Geometry: final body of the model. Coordinates: model frame, mm. A direction names the side the tool comes from. Give positions to 0.01 mm unless a question says otherwise; leave off trailing zeros. Order: outer loops, then holes, each group sorted by start corner. A loop starts at its lowest first (then second) coordinate and runs counter-clockwise, first axis right, second up. Notation, with made-up numbers: (-35.75, -19) - (17.25, -19) arc R14 cw to (17.25, -4) - close; hole circle Ø4 at (16, -9.5). An arc over 180 degrees is marked (long way). One line per item, written item: value.
```python
from build123d import *

# Parameters (mm, degrees)
SKETCH_1_W          = 80
SKETCH_1_H          = 50
EXTRUDE_1_DEPTH     = 1000
FILLET_1_R          = 5
SHELL_1_T           = -3
SKETCH_2_R          = 17.6
CUT_EXTRUDE_1_DEPTH = 1003.047903047
SKETCH_3_R          = 3.4
CUT_EXTRUDE_2_DEPTH = 10
SKETCH_4_R          = 2.5
CUT_EXTRUDE_3_DEPTH = 10


with BuildPart() as part:
    # 草图1 → 凸台-拉伸1 (new body)
    with BuildSketch(Plane.XY):
        Rectangle(SKETCH_1_W, SKETCH_1_H)
    extrude(amount=EXTRUDE_1_DEPTH)

    # 圆角1
    fillet_1_edges = [part.edges().sort_by_distance(p)[0] for p in [
        (40, -25, 500),
        (-40, -25, 500),
        (-40, 25, 500),
        (40, 25, 500),
    ]]
    fillet(fillet_1_edges, radius=FILLET_1_R)

    # 抽壳1
    shell_1_openings = [part.faces().sort_by_distance(p)[0] for p in [
        (0, 0, 1000),
        (0, 0, 0),
    ]]
    offset(amount=SHELL_1_T, openings=shell_1_openings, kind=Kind.INTERSECTION)

    # 草图2 → 切除-拉伸1 (cut, through all)
    with BuildSketch(Plane(origin=(0, 25, 0), x_dir=(1, 0, 0), z_dir=(0, 1, 0))):
        with Locations(Location((-4.7, -208, 0), (0, 0, 270))):
            Circle(SKETCH_2_R)
        with Locations(Location((-4.7, -792, 0), (0, 0, 270))):
            Circle(SKETCH_2_R)
    extrude(amount=-CUT_EXTRUDE_1_DEPTH, mode=Mode.SUBTRACT)

    # 草图3 → 切除-拉伸2 (cut)
    with BuildSketch(Plane(origin=(0, 25, 0), x_dir=(1, 0, 0), z_dir=(0, 1, 0))):
        with Locations(Location((15.3, -170.5, 0), (0, 0, 270))):
            Circle(SKETCH_3_R)
        with Locations(Location((-24.7, -170.5, 0), (0, 0, 270))):
            Circle(SKETCH_3_R)
        with Locations(Location((-24.7, -245.5, 0), (0, 0, 270))):
            Circle(SKETCH_3_R)
        with Locations(Location((15.3, -245.5, 0), (0, 0, 270))):
            Circle(SKETCH_3_R)
        with Locations(Location((15.3, -754.5, 0), (0, 0, 270))):
            Circle(SKETCH_3_R)
        with Locations(Location((-24.7, -754.5, 0), (0, 0, 270))):
            Circle(SKETCH_3_R)
        with Locations(Location((-24.7, -829.5, 0), (0, 0, 270))):
            Circle(SKETCH_3_R)
        with Locations(Location((15.3, -829.5, 0), (0, 0, 270))):
            Circle(SKETCH_3_R)
    extrude(amount=-CUT_EXTRUDE_2_DEPTH, mode=Mode.SUBTRACT)

    # 草图4 → 切除-拉伸3 (cut)
    with BuildSketch(Plane(origin=(0, 25, 0), x_dir=(1, 0, 0), z_dir=(0, 1, 0))):
        with Locations(Location((0, -475, 0), (0, 0, 270))):
            Circle(SKETCH_4_R)
        with Locations(Location((0, -500, 0), (0, 0, 270))):
            Circle(SKETCH_4_R)
    extrude(amount=-CUT_EXTRUDE_3_DEPTH, mode=Mode.SUBTRACT)


solid = part.part
```
1) Section A-A, the plane z = 792. Return loops of the section in (x, y), then the cut area to 3 significant figures.
Answers below:
outline: (-40, -20) arc R5 ccw to (-35, -25) - (-22.3, -25) - (-22.3, -22) - (-35, -22) arc R2 cw to (-37, -20) - (-37, 20) arc R2 cw to (-35, 22) - (-22.3, 22) - (-22.3, 25) - (-35, 25) arc R5 ccw to (-40, 20) - close; (12.9, -25) - (35, -25) arc R5 ccw to (40, -20) - (40, 20) arc R5 ccw to (35, 25) - (12.9, 25) - (12.9, 22) - (35, 22) arc R2 cw to (37, 20) - (37, -20) arc R2 cw to (35, -22) - (12.9, -22) - close
area: 515 mm^2
2) Section C-C, the plane z = 97. Return loops of the section in (x, y).
Answers below:
outline: (-40, -20) arc R5 ccw to (-35, -25) - (35, -25) arc R5 ccw to (40, -20) - (40, 20) arc R5 ccw to (35, 25) - (-35, 25) arc R5 ccw to (-40, 20) - close; hole (-37, -20) arc R2 ccw to (-35, -22) - (35, -22) arc R2 ccw to (37, -20) - (37, 20) arc R2 ccw to (35, 22) - (-35, 22) arc R2 ccw to (-37, 20) - close
3) Mould query, pull axis X, two halves, no side actions, for faces 1 (the face through (-40, 0, 493)), 2 (the face through (-0.2, 22.3, 0)), 3 (the face through (40, 0, 493)), 4 (the face through (-37, 0, 493)). Classes: released by +X, released by -X, zero draft, split by the parting line, or undercut.
Answers below:
face 1: released by -X
face 2: zero draft
face 3: released by +X
face 4: undercut
4) Set-up query: faces 5 (the face through (-3.926, -23.479, 774.417)), 6 (the face through (0, 22, 493)). Return all of +Z, -Z, +X, -X, +Y, -Y with unobstructed straight access to the full face (end or side cutting, diameter ignored); none if empty.
Answers below:
face 5: +Y, -Y
face 6: +Z, -Z
5) Material intervals for line 1 along X through (y, z) = (20, 478); line 2 along Y through (x, z) = (-23, 84.5); line 3 along X through (y, z) = (23, 245), sorted ascending.
Answers below:
line 1: -40 to -37, 37 to 40
line 2: -25 to -22, 22 to 25
line 3: -39 to -28.06, -21.34 to 11.94, 18.66 to 39
6) First-contact query: pin 1 (11 mm diameter, centred on x = -24.7, z = 170.5, fed in from +Y); pin 2 (21 mm diameter, centred on x = -4.7, z = 208, fed in from +Y); pin 3 (4 mm diameter, centred on x = 15.3, z = 754.5, fed in from +Y). Flat tips, straight axial feed; report the tip coordinate or a pass-through.
Answers below:
pin 1: y = 25
pin 2: through
pin 3: y = -22
7) Section B-B, the plane y = -5.5. Return loops of the section in (x, z).
Answers below:
outline: (-40, 0) - (-37, 0) - (-37, 1000) - (-40, 1000) - close; (37, 0) - (40, 0) - (40, 1000) - (37, 1000) - close
